from build123d import *

# Parameters (mm, degrees)
BOSS_EXTRU_1_DEPTH = 2


with BuildPart() as part:
    # Sketch1 → Boss.-Extru.1 (new body)
    with BuildSketch(Plane(origin=(0, 0, 0), x_dir=(1, 0, 0), z_dir=(0, 1, 0))):
        with BuildLine():
            Line((8.5, 17.5), (-8.5, 17.5))
            ThreePointArc((-8.5, 17.5), (-11.328427125, 16.328427125), (-12.5, 13.5))
            Line((-12.5, 13.5), (-12.5, -13.5))
            ThreePointArc((-12.5, -13.5), (-11.328427125, -16.328427125), (-8.5, -17.5))
            Line((-8.5, -17.5), (8.5, -17.5))
            ThreePointArc((8.5, -17.5), (11.328427125, -16.328427125), (12.5, -13.5))
            Line((12.5, -13.5), (12.5, 13.5))
            ThreePointArc((12.5, 13.5), (11.328427125, 16.328427125), (8.5, 17.5))
        make_face()
    extrude(amount=BOSS_EXTRU_1_DEPTH)


solid = part.part
Check sheet for the modelled part. Datum: model origin and axes. Units: mm. Give positions to 0.01 mm unless a question says otherwise; leave off trailing zeros. Write each loop counter-clockwise with the first axis right and the second up, starting at its lowest first coordinate (ties: lowest second). Pieces come first, ordered by that corner, then holes. Notation, with made-up numbers: (-27, 25.5) -> (29, 25.5) arc R31 cw to (29, 62.5) -> close; hole circle Ø2 at (-36.5, 41). An arc over 180 degrees is marked (long way). One line per item, written item: value. Start each with the question number.
Item 1: Gauge pin test, flat ends, axial feed: pin 1 (1 mm diameter, centred on x = -9.5, y = 0.5, fed in from +Z); pin 2 (12 mm diameter, centred on x = 10, z = 2, fed in from -Y). Record the tip position at first contact, or that the pin passes through.
Item 2: Section check A-A on y = 0.65. Record the cut outline in (x, z).
Item 3: Material ranges on probe 1 along Z at (x, y) = (-8.75, 1.1); probe 2 along Z at (x, y) = (-11.25, 0.85); probe 3 along X at (y, z) = (1.5, 15), recorded low to high. Write a range as from..to.
Results list:
1. pin 1: z = 17.47
1. pin 2: y = 0
2. outline: (-12.5, -13.5) arc R4 ccw to (-8.5, -17.5) -> (8.5, -17.5) arc R4 ccw to (12.5, -13.5) -> (12.5, 13.5) arc R4 ccw to (8.5, 17.5) -> (-8.5, 17.5) arc R4 ccw to (-12.5, 13.5) -> close
3. probe 1: -17.49..17.49
3. probe 2: -16.4..16.4
3. probe 3: -12.21..12.21
